Geometry check sheet. Reference: the model listing, model coordinates, mm. Face numbers are marked on the shaded views. A direction names the side the tool comes from. Round coordinates to 2 decimals unless told otherwise and drop trailing zeros. Write each loop counter-clockwise with the first axis right and the second up, starting at its lowest first coordinate (ties: lowest second). Pieces come first, ordered by that corner, then holes. Notation, with made-up numbers: M 19.25,85 L 23.25,85 A26 cw 23.25,109 Z; hole C 18,83.25 d10. An arc over 180 degrees is marked long. One line per item, written item: value. Start each with the question number.
1. Depth check by flat-ended pin: P1, Ø0.7, axis at y = -12, z = 2, coming from the +X side; P2, Ø1.2, axis at y = -4, z = -9.5, coming from the +X side; P3, Ø8, axis at x = 53.5, z = -7, coming from the +Y side. Enter the tip coordinate at first touch or a pass-through.
2. Scan lines: probe 1 along X at (y, z) = (-1.75, 8); probe 2 along Z at (x, y) = (82.5, 1.5); probe 3 along Y at (x, z) = (55, 5.75). Record each from-to range of solid material in increasing order. Write a range as [from, to].
3. Section check A-A (x = 7.5). Record the boundary of the cut face in (y, z) (3 decimals).
4. Access from +Z, -Z, +X, -X, +Y, -Y to the whole of each face (thin tool, end or side, straight path). Record for the marked faces 1 and 2.
5. Section check B-B (x = 45). Record the boundary of the cut face in (y, z), and give its area (3 significant figures).
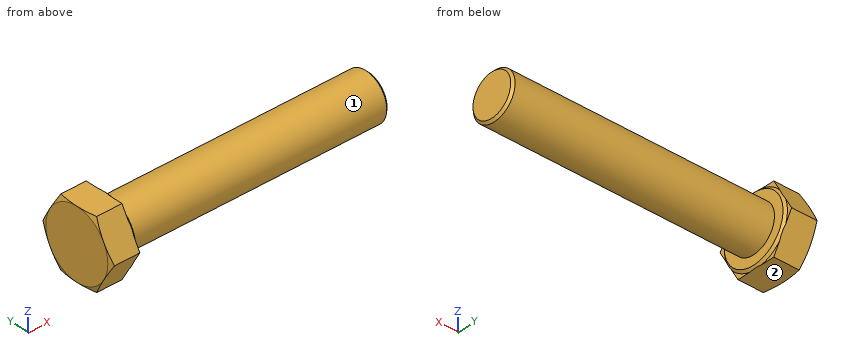
from build123d import *

# Parameters (mm, degrees)
BASEHEAD_DEPTH = 10.18
SKETCH5_R      = 8
BASEBODY_DEPTH = 90
CHAMFER1_SIZE  = 0.8


with BuildPart() as part:
    # Sketch2 → BaseHead (new body)
    with BuildSketch(Plane(origin=(0, 0, 0), x_dir=(0, 0, -1), z_dir=(1, 0, 0))):
        Polygon((11.835, -6.832940436), (11.835, 6.832940436), (0, 13.665880872), (-11.835, 6.832940436), (-11.835, -6.832940436), (0, -13.665880872), align=None)
    extrude(amount=BASEHEAD_DEPTH)

    # Sketch3 → BearingFace (revolve, cut)
    with BuildSketch(Plane.XY, mode=Mode.PRIVATE) as bearingface_sk:
        Polygon((10.18, 13.665880872), (10.18, 11.245), (9.38, 12.045), (9.38, 13.665880872), align=None)
    revolve(bearingface_sk.sketch.rotate(Axis((-0.957090588, 0, 0), (1, 0, 0)), 90), axis=Axis((-0.957090588, 0, 0), (1, 0, 0)), mode=Mode.SUBTRACT)

    # Sketch4 → Head chamfer (revolve, cut)
    with BuildSketch(Plane.XY):
        Polygon((0, 13.665880872), (0.66638614, 13.665880872), (0, 11.835), align=None)
    revolve(axis=Axis((-0.493528746, 0, 0), (1, 0, 0)), mode=Mode.SUBTRACT)

    # Sketch5 → BaseBody (add)
    with BuildSketch(Plane(origin=(10.18, 0, 0), x_dir=(0, 0, -1), z_dir=(1, 0, 0))):
        with Locations(Location((0, 0, 0), (0, 0, 180))):
            Circle(SKETCH5_R)
    extrude(amount=BASEBODY_DEPTH)

    # Chamfer1
    chamfer1_edges = [part.edges().sort_by_distance(p)[0] for p in [
        (100.18, 0, -8),
    ]]
    chamfer(chamfer1_edges, length=CHAMFER1_SIZE)


solid = part.part
Result sheet:
1. P1: stops at x = 9.61
1. P2: stops at x = 10.18
1. P3: stops at y = 7.42
2. probe 1: x = [0, 10.18]
2. probe 2: z = [-7.86, 7.86]
2. probe 3: y = [-5.56, 5.56]
3. outline: M -13.666,0 L -6.833,-11.835 L 6.833,-11.835 L 13.666,0 L 6.833,11.835 L -6.833,11.835 Z
4. face 1: +X
4. face 2: -Z, +X, -X, +Y, -Y
5. outline: C 0,0 d16
5. area: 201 mm2
